```python
from build123d import *

# Parameters (mm, degrees)
SKETCH3_R          = 2.75
CUT_EXTRUDE2_DEPTH = 4
SKETCH4_R          = 4
CUT_EXTRUDE3_DEPTH = 10
SKETCH5_W          = 5.699016122
SKETCH5_H          = 1.5


with BuildPart() as part:
    # Sketch1 → Revolve1 (revolve)
    with BuildSketch(Plane.XY):
        Polygon((-8.5, -6.487039895), (-8.5, -15.445084434), (-4, -19.945084434), (0, -19.945084434), (0, 12.633854157), (0, 15.364763468), (-5.101647841, 15.364763468), (-5.101647841, 14.4706398), (-4.341150579, 14.4706398), (-4.341150579, 12.633854157), (-5.101647841, 12.633854157), (-5.101647841, 6.827224241), (-3.580653318, 3.948464428), (-3.580653318, 2.293177536), (-4.341150579, 1.532680274), (-4.341150579, -6.487039895), align=None)
    revolve(axis=Axis((0, 12.633854157, 0), (0, -1, 0)))

    # Sketch3 → Cut-Extrude2 (cut)
    with BuildSketch(Plane(origin=(0, 15.364763468, 0), x_dir=(1, 0, 0), z_dir=(0, 1, 0))):
        with Locations(Location((0, 0, 0), (0, 0, 180))):
            Circle(SKETCH3_R)
    extrude(amount=-CUT_EXTRUDE2_DEPTH, mode=Mode.SUBTRACT)

    # Sketch4 → Cut-Extrude3 (cut)
    with BuildSketch(Plane.XZ.offset(19.945084434)):
        Circle(SKETCH4_R)
    extrude(amount=-CUT_EXTRUDE3_DEPTH, mode=Mode.SUBTRACT)

    # Sketch5 → Cut-Revolve1 (revolve, cut)
    with BuildSketch(Plane(origin=(0, 0, 0), x_dir=(0, 0, -1), z_dir=(1, 0, 0)), mode=Mode.PRIVATE) as cut_revolve1_sk:
        with Locations((6.332308204, -16.695084434)):
            Rectangle(SKETCH5_W, SKETCH5_H)
    cut_revolve1 = revolve(cut_revolve1_sk.sketch.rotate(Axis((0, -17.445084434, -3.482800143), (0, 0, -1)), 90), axis=Axis((0, -17.445084434, -3.482800143), (0, 0, -1)), mode=Mode.SUBTRACT)

    # Mirror1: Cut-Revolve1 across plane
    add(cut_revolve1.mirror(Plane.XY), mode=Mode.SUBTRACT)


solid = part.part
```
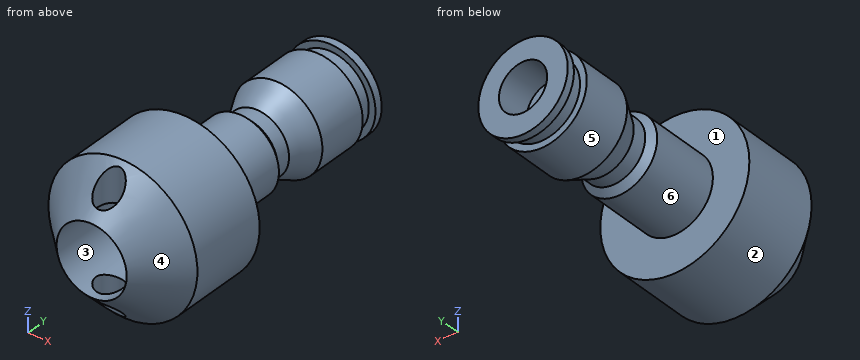
For this review, take the finished solid that the model builds, in its own axes (mm). Face numbers are marked on the shaded views. A direction names the side the tool comes from. Round coordinates to 2 decimals unless told otherwise and drop trailing zeros. Order: outer loops, then holes, each group sorted by start corner. A loop starts at its lowest first (then second) coordinate and runs counter-clockwise, first axis right, second up.
Q1. Wall thickness on line 1 (X direction, y = -14.25, z = 0); line 2 (Z direction, x = 0, y = 12.35); line 3 (Z direction, x = 0, y = 12.9): over which ranges is each line inside the solid? List them lowest first.
Findings below:
line 1: x = -8.5 to -4, 4 to 8.5
line 2: z = -5.1 to -2.75, 2.75 to 5.1
line 3: z = -4.34 to -2.75, 2.75 to 4.34
Q2. We need section A-A, the plane x = 0. State how many separate pieces and enclosed holes the cut face has, plus the area to 3 significant figures.
Findings below:
separate pieces: 3
enclosed holes: 0
area: 288 mm2
Q3. Machinability: for the marked faces 4, 5 and 6, which of the approach directions +Z, -Z, +X, -X, +Y, -Y give a long, thin tool a straight path to every point of the face, cutting with its end or side? Answer none if there is none.
Findings below:
face 4: -Y
face 5: +Y
face 6: none
Q4. We need section C-C, the plane y = -8. Give the boundary of the cut face in (x, z).
Findings below:
outline: circle Ø17 at (0, 0)
Q5. Insertion check: P1, Ø3, axis at x = 0, z = -0.5, coming from the +Y side; P2, Ø2, axis at x = -6.5, z = -1, coming from the -Y side; P3, Ø3, axis at y = -13, z = 5.5, coming from the -X side. Each pin has a flat end and moves straight along its axis. Give the tip position at first contact, or say it passes through.
Findings below:
P1: stops at y = 11.36
P2: stops at y = -18.37
P3: stops at x = -7.5
Q6. Mouldability with a two-part tool opening along Z and no side actions: class the marked faces 1, 2 and 3 as pulls with the +Z half, pulls with the -Z half, needs draft (parallel to the pull), parting line crosses it, or undercut.
Findings below:
face 1: needs draft
face 2: parting line crosses it
face 3: undercut
